```python
from build123d import *

# Parameters (mm, degrees)
SKETCH1_W           = 13.4
SKETCH1_H           = 26
BOSS_EXTRUDE1_DEPTH = 6.4
SKETCH2_W           = 5
SKETCH2_H           = 9
CUT_EXTRUDE1_DEPTH  = 30.941943825
SKETCH3_W           = 26
SKETCH3_H           = 6.2
BOSS_EXTRUDE2_DEPTH = 3
CUT_EXTRUDE2_DEPTH  = 34.436506995
SKETCH5_W           = 13.4
SKETCH5_H           = 3.2
CUT_EXTRUDE3_DEPTH  = 0.5
SKETCH6_W           = 13.4
SKETCH6_H           = 3.2
CUT_EXTRUDE4_DEPTH  = 0.5
SKETCH7_W           = 2
SKETCH7_H           = 9.197470194
BOSS_EXTRUDE3_DEPTH = 0.2
LPATTERN1_COUNT     = 4
LPATTERN1_PITCH     = 3


with BuildPart() as part:
    # Sketch1 → Boss-Extrude1 (new body)
    with BuildSketch(Plane.XY):
        with Locations((-6.7, 13)):
            Rectangle(SKETCH1_W, SKETCH1_H)
    extrude(amount=BOSS_EXTRUDE1_DEPTH)

    # Sketch2 → Cut-Extrude1 (cut, through all)
    with BuildSketch(Plane.XY.offset(6.4)):
        with Locations((-6.7, 21.5)):
            Rectangle(SKETCH2_W, SKETCH2_H)
    extrude(amount=-CUT_EXTRUDE1_DEPTH, mode=Mode.SUBTRACT)

    # Sketch3 → Boss-Extrude2 (add)
    with BuildSketch(Plane.ZY.offset(13.4)):
        with Locations((3.2, 6.3)):
            Rectangle(SKETCH3_W, SKETCH3_H)
    extrude(amount=-BOSS_EXTRUDE2_DEPTH)

    # Sketch4 → Cut-Extrude2 (cut, through all)
    with BuildSketch(Plane.ZY.offset(13.4)):
        with BuildLine():
            Line((-6.8, 7.9), (-5.9, 7.9))
            ThreePointArc((-5.9, 7.9), (-4.3, 6.3), (-5.9, 4.7))
            Line((-5.9, 4.7), (-6.8, 4.7))
            ThreePointArc((-6.8, 4.7), (-8.4, 6.3), (-6.8, 7.9))
        make_face()
        with BuildLine():
            Line((13.2, 7.9), (14.1, 7.9))
            ThreePointArc((14.1, 7.9), (15.7, 6.3), (14.1, 4.7))
            Line((14.1, 4.7), (13.2, 4.7))
            ThreePointArc((13.2, 4.7), (11.6, 6.3), (13.2, 7.9))
        make_face()
    extrude(amount=-CUT_EXTRUDE2_DEPTH, mode=Mode.SUBTRACT)

    # Sketch5 → Cut-Extrude3 (cut)
    with BuildSketch(Plane.XY.offset(6.4)):
        with Locations((-6.7, 1.6)):
            Rectangle(SKETCH5_W, SKETCH5_H)
    extrude(amount=-CUT_EXTRUDE3_DEPTH, mode=Mode.SUBTRACT)

    # Sketch6 → Cut-Extrude4 (cut)
    with BuildSketch(Plane(origin=(0, 0, 0), x_dir=(-1, 0, 0), z_dir=(0, 0, -1))):
        with Locations((6.7, 1.6)):
            Rectangle(SKETCH6_W, SKETCH6_H)
    extrude(amount=-CUT_EXTRUDE4_DEPTH, mode=Mode.SUBTRACT)

    # Sketch7 → Boss-Extrude3 (add)
    with BuildSketch(Plane.XY.offset(5.9)):
        with Locations((-2.2, -1.958933194)):
            Rectangle(SKETCH7_W, SKETCH7_H)
    boss_extrude3 = extrude(amount=BOSS_EXTRUDE3_DEPTH)

    # LPattern1: Boss-Extrude3 ×4
    with Locations(*[(-i * LPATTERN1_PITCH, 0, 0) for i in range(1, LPATTERN1_COUNT)]):
        add(boss_extrude3)


solid = part.part
```
CAD build for the part. Positions are in the model's coordinates, mm. A direction names the side the tool comes from. Round coordinates to 2 decimals unless told otherwise and drop trailing zeros. Write each loop counter-clockwise with the first axis right and the second up, starting at its lowest first coordinate (ties: lowest second). Pieces come first, ordered by that corner, then holes.
Item 1: Band-saw the part on B-B on y = 18.5. Write the cut outline in (x, z), then the cut area to 3 significant figures.
Filled in:
outline: (-13.4, 0) - (-9.2, 0) - (-9.2, 6.4) - (-13.4, 6.4) - close; (-4.2, 0) - (0, 0) - (0, 6.4) - (-4.2, 6.4) - close
area: 53.8 mm2
Item 2: Band-saw the part on A-A on y = -3. Write the cut outline in (x, z).
Filled in:
outline: (-12.2, 5.9) - (-10.2, 5.9) - (-10.2, 6.1) - (-12.2, 6.1) - close; (-9.2, 5.9) - (-7.2, 5.9) - (-7.2, 6.1) - (-9.2, 6.1) - close; (-6.2, 5.9) - (-4.2, 5.9) - (-4.2, 6.1) - (-6.2, 6.1) - close; (-3.2, 5.9) - (-1.2, 5.9) - (-1.2, 6.1) - (-3.2, 6.1) - close
Item 3: Drill centre lines: L1, parallel to Z at x = -2.5, y = 20; L2, parallel to Y at x = -2.25, z = 2.75; L3, parallel to Y at x = -12.5, z = 7.25. Where is each one in solid material? Low to high.
Filled in:
L1: z = 0 to 6.4
L2: y = 0 to 26
L3: y = 3.2 to 9.4
Item 4: Mould opens along Z. For faces 6 (the flat face through (-11.9, 4.7, 13.7)), 7 (the flat face through (-2, -3, 5.9)), 8 (the flat face through (-12, 9.4, 11)) say: released by +Z, released by -Z, zero draft, split by the parting line, or undercut.
Filled in:
face 6: undercut
face 7: released by -Z
face 8: zero draft
Item 5: Band-saw the part on D-D on y = 9. Write the cut outline in (x, z).
Filled in:
outline: (-13.4, -9.8) - (-10.4, -9.8) - (-10.4, 0) - (0, 0) - (0, 6.4) - (-10.4, 6.4) - (-10.4, 16.2) - (-13.4, 16.2) - close
Item 6: Tool access for faces 1 (the cylindrical face through (-11.9, 6.3, -4.3)), 2 (the flat face through (-10.4, 6, 10)), 3 (the flat face through (-11, -2, 6.1)), 4 (the flat face through (-4.2, 21, 3)), 5 (the flat face through (-5, -3, 5.9)): list every direction of +Z, -Z, +X, -X, +Y, -Y with a clear straight run to the whole face (end or side of a thin tool).
Filled in:
face 1: +X, -X
face 2: +Z, +X, +Y, -Y
face 3: +Z, +X, -X, -Y
face 4: +Z, -Z, +Y
face 5: -Z, +X, -X, -Y
Item 7: Band-saw the part on C-C on x = -3.75. Write the cut outline in (y, z).
Filled in:
outline: (0, 0.5) - (3.2, 0.5) - (3.2, 0) - (26, 0) - (26, 6.4) - (3.2, 6.4) - (3.2, 5.9) - (0, 5.9) - close
Item 8: Drop flat-ended pins along their axis: pin 1 Ø1 at (x, y) = (-5, -2) entering from +Z; pin 2 Ø0.7 at (x, z) = (-12, 13.5) entering from -Y; pin 3 Ø2 at (x, y) = (-2, -2.5) entering from -Z; pin 4 Ø1.5 at (x, z) = (-2.5, -1.5) entering from -Y. Give the stop position or say it passes through.
Filled in:
pin 1: stops at z = 6.1
pin 2: stops at y = 3.2
pin 3: stops at z = 5.9
pin 4: passes through
